Geometry: final body of the model. Coordinates: model frame, mm. A direction names the side the tool comes from. Give positions to 0.01 mm unless a question says otherwise; leave off trailing zeros. Loops run counter-clockwise (first coordinate to the right, second up) from the corner with the lowest first, then second, coordinate; pieces in that order, holes last.
1. Section C-C, the plane x = 4.75. Output: boundary loops of the cut face in (y, z).
2. Section B-B, the plane y = -15. Output: boundary loops of the cut face in (x, z).
3. Material intervals for line 1 along Y through (x, z) = (21.75, 320); line 2 along X through (y, z) = (-21.25, 85), sorted ascending.
4. Access query for faces 1 (the face through (30, -15, 242)), 2 (the face through (12, -4, 242)). Directions: +Z, -Z, +X, -X, +Y, -Y. A direction counts if a zero-diameter tool reaches every point of the face in a straight line with its end or side. Return the directions, or none.
5. First-contact query: P1, Ø1, axis at x = 11.5, z = 357, coming from the -Y side; P2, Ø12, axis at y = -13, z = 365, coming from the -X side. Flat tips, straight axial feed; report the tip coordinate or a pass-through.
6. Section A-A, the plane z = 313. Output: boundary loops of the cut face in (x, y).
from build123d import *

# Parameters (mm, degrees)
BOSS_EXTRUDE1_DEPTH = 490


with BuildPart() as part:
    # Sketch1 → Boss-Extrude1 (new body)
    with BuildSketch(Plane.XY):
        with BuildLine():
            Line((0, 0), (30, 0))
            Line((30, 0), (30, -30))
            Line((30, -30), (26, -30))
            Line((26, -30), (26, -6))
            ThreePointArc((26, -6), (25.414213562, -4.585786438), (24, -4))
            Line((24, -4), (0, -4))
            Line((0, -4), (0, 0))
        make_face()
    extrude(amount=BOSS_EXTRUDE1_DEPTH)


solid = part.part
Answers below:
1. outline: (-4, 0) - (0, 0) - (0, 490) - (-4, 490) - close
2. outline: (26, 0) - (30, 0) - (30, 490) - (26, 490) - close
3. line 1: y = -4 to 0
3. line 2: x = 26 to 30
4. face 1: +Z, -Z, +X, +Y, -Y
4. face 2: +Z, -Z, -X, -Y
5. P1: stops at y = -4
5. P2: stops at x = 26
6. outline: (0, -4) - (24, -4) arc R2 cw to (26, -6) - (26, -30) - (30, -30) - (30, 0) - (0, 0) - close
